from build123d import *

# Parameters (mm, degrees)
SKETCH1_R           = 5
BOSS_EXTRUDE1_DEPTH = 15
BOSS_EXTRUDE2_START = 35
SKETCH2_R           = 5
BOSS_EXTRUDE2_DEPTH = 35
CUT_EXTRUDE1_DEPTH  = 3.5
SKETCH5_R           = 5
SKETCH5_R_2         = 3.5
CUT_EXTRUDE2_DEPTH  = 5.3
CHAMFER1_SIZE       = 1


with BuildPart() as part:
    # Sketch1 → Boss-Extrude1 (new body)
    with BuildSketch(Plane(origin=(0, 0, 0), x_dir=(1, 0, 0), z_dir=(0, 1, 0))):
        with Locations(Location((0, 0, 0), (0, 0, 270))):
            Circle(SKETCH1_R)
    extrude(amount=BOSS_EXTRUDE1_DEPTH)

    # Sketch2 → Boss-Extrude2 (add)
    with BuildSketch(Plane.XZ.offset(BOSS_EXTRUDE2_START)):
        with Locations(Location((0, 0, 0), (0, 0, 270))):
            Circle(SKETCH2_R)
    extrude(amount=-BOSS_EXTRUDE2_DEPTH)

    # Sketch3 → Cut-Extrude1 (cut)
    with BuildSketch(Plane(origin=(0, 15, 0), x_dir=(1, 0, 0), z_dir=(0, 1, 0))):
        Polygon((0, 2.8615), (-2.478131693, 1.43075), (-2.478131693, -1.43075), (0, -2.8615), (2.478131693, -1.43075), (2.478131693, 1.43075), align=None)
    extrude(amount=-CUT_EXTRUDE1_DEPTH, mode=Mode.SUBTRACT)

    # Sketch4 → Cut-Revolve1 (revolve, cut)
    with BuildSketch(Plane.XY, mode=Mode.PRIVATE) as cut_revolve1_sk:
        Polygon((0, 11.5), (2.478131693, 11.5), (0, 10.06925), align=None)
        Polygon((2.478131693, 14.778662205), (2.478131693, 15), (2.8615, 15), align=None)
    revolve(cut_revolve1_sk.sketch.rotate(Axis((0, -3.932195077, 0), (0, 1, 0)), 90), axis=Axis((0, -3.932195077, 0), (0, 1, 0)), mode=Mode.SUBTRACT)

    # Sketch5 → Cut-Extrude2 (cut)
    with BuildSketch(Plane.XZ.offset(35)):
        with Locations(Location((0, 0, 0), (0, 0, 270))):
            Circle(SKETCH5_R)
        with Locations(Location((0, 0, 0), (0, 0, 270))):
            Circle(SKETCH5_R_2, mode=Mode.SUBTRACT)
    extrude(amount=-CUT_EXTRUDE2_DEPTH, mode=Mode.SUBTRACT)

    # Chamfer1
    chamfer1_edges = [part.edges().sort_by_distance(p)[0] for p in [
        (0, 15, -5),
        (0, -29.7, 5),
    ]]
    chamfer(chamfer1_edges, length=CHAMFER1_SIZE)


solid = part.part
Here's how the part is built. I have some questions about the finished solid (model axes, mm). A direction names the side the tool comes from. Give positions to 0.01 mm unless a question says otherwise; leave off trailing zeros. Order: outer loops, then holes, each group sorted by start corner. A loop starts at its lowest first (then second) coordinate and runs counter-clockwise, first axis right, second up. Notation, with made-up numbers: (67, -29.5) -> (106, -29.5) arc R20 cw to (106, 9.5) -> close; hole circle Ø3 at (-24, 10). An arc over 180 degrees is marked (long way). One line per item, written item: value. Start each with the question number.
1. We'd pull the mould along Z, two halves only. Please class faces 3 (the face through (-3.417, -32.387, 0.759)), 4 (the face through (2.3, 11.5, 1.3)), 5 (the face through (0, -35, 0)): released by +Z, released by -Z, zero draft, split by the parting line, or undercut.
2. Imagine slicing it at B-B, the plane y = -31. List the corners of the cut face in (x, z) for me.
3. For faces 1 (the face through (1.35, 14.888, -2.3)), 2 (the face through (3, 15, -1)), which set-ups out of +Z, -Z, +X, -X, +Y, -Y let a thin tool reach every point of the face, with its end or its side?
4. Will these pins go through, and if not, where does the flat tip stop? pin 1 Ø2 at (x, y) = (-2, -22) entering from +Z; pin 2 Ø1 at (x, z) = (-1.5, 1.5) entering from +Y; pin 3 Ø0.6 at (x, z) = (-2, -1) entering from +Y.
5. Imagine slicing it at A-A, the plane y = 6. List the corners of the cut face in (x, z) for me, plus the area to 3 significant figures.
6. I need wall thicknesses on probe 1 along X at (y, z) = (-28.5, -0.25); probe 2 along X at (y, z) = (13.5, -2); probe 3 along Y at (x, z) = (-0.25, 0.75). Which ranges of each line are inside material? Lowest first, please. Write a range as from..to.
Values follow:
1. face 3: split by the parting line
1. face 4: undercut
1. face 5: zero draft
2. outline: circle Ø7 at (0, 0)
3. face 1: +Y
3. face 2: +Z, -Z, +X, -X, +Y
4. pin 1: stops at z = 4.9
4. pin 2: stops at y = 14.86
4. pin 3: stops at y = 11.5
5. outline: circle Ø10 at (0, 0)
5. area: 78.5 mm2
6. probe 1: x = -4.99..4.99
6. probe 2: x = -4.58..-1.49, 1.49..4.58
6. probe 3: y = -35..10.53
